Build history of the part. All positions in model axes, mm. Coordinates: 2 decimals unless noted, no trailing zeros. Order: outer loops, then holes, each group sorted by start corner. A loop starts at its lowest first (then second) coordinate and runs counter-clockwise, first axis right, second up. Notation, with made-up numbers: (-7.5, 31.25) - (19.5, 31.25) arc R20 ccw to (19.5, 45.25) - close; hole circle Ø3 at (12, 80.5). An arc over 180 degrees is marked (long way). Return JSON: item names as keys, results as strings.
from build123d import *

# Parameters (mm, degrees)
SKETCH_1_R          = 20.25
EXTRUDE_1_DEPTH     = 100
SKETCH_2_R          = 14
CUT_EXTRUDE_1_DEPTH = 8
SKETCH_3_R          = 12.5
CUT_EXTRUDE_2_DEPTH = 195.12399388
CHAMFER_1_SIZE      = 0.5


with BuildPart() as part:
    # 草图1 → 凸台-拉伸1 (new, symmetric)
    with BuildSketch(Plane.XY):
        Circle(SKETCH_1_R)
    extrude(amount=EXTRUDE_1_DEPTH, both=True)

    # 草图2 → 切除-拉伸1 (cut)
    with BuildSketch(Plane.XY.offset(100)):
        Circle(SKETCH_2_R)
    cut_extrude_1 = extrude(amount=-CUT_EXTRUDE_1_DEPTH, mode=Mode.SUBTRACT)

    # 镜向1: 切除-拉伸1 across plane
    add(cut_extrude_1.mirror(Plane.XY), mode=Mode.SUBTRACT)

    # 草图3 → 切除-拉伸2 (cut, through all)
    with BuildSketch(Plane.XY.offset(92)):
        Circle(SKETCH_3_R)
    extrude(amount=-CUT_EXTRUDE_2_DEPTH, mode=Mode.SUBTRACT)

    # 倒角1
    chamfer_1_edges = [part.edges().sort_by_distance(p)[0] for p in [
        (-14, 0, -100),
        (-20.25, 0, -100),
        (-20.25, 0, 100),
        (-14, 0, 100),
    ]]
    chamfer(chamfer_1_edges, length=CHAMFER_1_SIZE)


solid = part.part
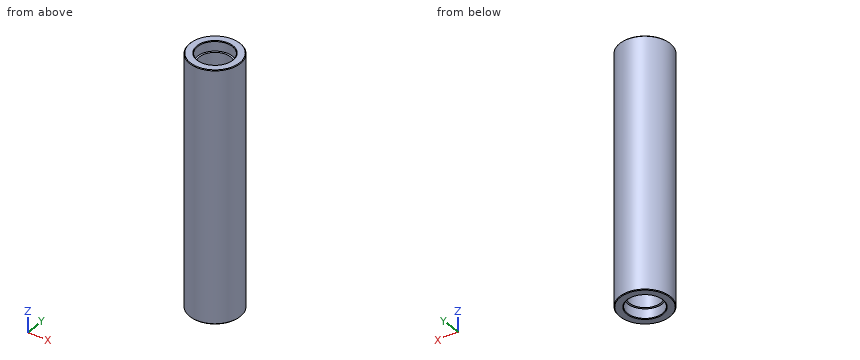
1. Drop flat-ended pins along their axis: pin 1 (10 mm diameter, centred on x = 14.5, z = -49, fed in from +Y); pin 2 (12 mm diameter, centred on x = 8.5, z = -4, fed in from +Y); pin 3 (12 mm diameter, centred on x = 7.5, z = 65.5, fed in from +Y); pin 4 (10 mm diameter, centred on y = -4, z = 61.5, fed in from -X). Give the stop position or say it passes through.
Check values:
{"pin 1": "y = 17.88", "pin 2": "y = 20.1", "pin 3": "y = 20.19", "pin 4": "x = -20.25"}
2. Cut at A-A on x = 0. Give the cut face in (y, z).
Check values:
{"outline": "(-20.25, -99.5) - (-19.75, -100) - (-14.5, -100) - (-14, -99.5) - (-14, -92) - (-12.5, -92) - (-12.5, 92) - (-14, 92) - (-14, 99.5) - (-14.5, 100) - (-19.75, 100) - (-20.25, 99.5) - close; (12.5, -92) - (14, -92) - (14, -99.5) - (14.5, -100) - (19.75, -100) - (20.25, -99.5) - (20.25, 99.5) - (19.75, 100) - (14.5, 100) - (14, 99.5) - (14, 92) - (12.5, 92) - close"}
3. Probe L1, parallel to X at y = -1, z = -54.5; L2, parallel to Y at x = 0, z = -93.5; L3, parallel to Y at x = 0, z = -25. List the from-to ranges inside material, lowest first.
Check values:
{"L1": "-20.23 to -12.46, 12.46 to 20.23", "L2": "-20.25 to -14, 14 to 20.25", "L3": "-20.25 to -12.5, 12.5 to 20.25"}
4. Cut at C-C on z = 77. Give the cut face in (x, y).
Check values:
{"outline": "circle Ø40.5 at (0, 0); hole circle Ø25 at (0, 0)"}
